from build123d import *

# Parameters (mm, degrees)
CUT_EXTRUDE1_DEPTH      = 16
CUT_EXTRUDE1_DEPTH_BACK = 16


with BuildPart() as part:
    # Sketch1 → Revolve1 (revolve)
    with BuildSketch(Plane.XY, mode=Mode.PRIVATE) as revolve1_sk:
        Polygon((7.91882362, 0), (6, 3.3235), (-6.3235, 3.3235), (-7, 4), (-7, 8), (30, 8), (30, 16), (35, 16), (35, 0), align=None)
    revolve(revolve1_sk.sketch.rotate(Axis((35, 0, 0), (-1, 0, 0)), 270), axis=Axis((35, 0, 0), (-1, 0, 0)))

    # Sketch2 → Cut-Extrude1 (cut, two sides: drawn at the far end of the back side and taken through both)
    with BuildSketch(Plane(origin=(0, 0, 0), x_dir=(1, 0, 0), z_dir=(0, 1, 0)).offset(-CUT_EXTRUDE1_DEPTH_BACK)):
        Polygon((-12, 12), (-12, -12), (4.5, -12), (-0.5, -7), (-7, -7), (-7, 7), (-0.5, 7), (4.5, 12), align=None)
    extrude(amount=CUT_EXTRUDE1_DEPTH + CUT_EXTRUDE1_DEPTH_BACK, mode=Mode.SUBTRACT)


solid = part.part
Could you check a few things on this model? Use its own coordinates, in mm. A direction names the side the tool comes from. Coordinates: 2 decimals unless noted, no trailing zeros. Write each loop counter-clockwise with the first axis right and the second up, starting at its lowest first coordinate (ties: lowest second). Pieces come first, ordered by that corner, then holes. Notation, with made-up numbers: (-9.5, 26.5) - (37.5, 26.5) arc R27 cw to (37.5, 49.5) - close; hole circle Ø6 at (60, -20). An arc over 180 degrees is marked (long way). Put each result on its own line as item: value. Start each with the question number.
Q1. I want a section at A-A on z = -5. Write out the boundary of the cut face in (x, y) (3 decimals).
Q2. Which directions (+Z, -Z, +X, -X, +Y, -Y) give clear straight access to the entire face, cutting with the end or side of a thin tool? Please do faces 1 (the flat face through (35, 0, 0)), 2 (the flat face through (-7, 4, 2)), 3 (the flat face through (-4, 0, 7)), 4 (the cylindrical face through (12, 0, -8)), 5 (the flat face through (-4, 0, -7)).
Q3. Thinking about a two-plate mould opening in Y: for faces 6 (the cylindrical face through (32.53, -15.62, -3.47)), 7 (the flat face through (30, 7.3, 3.8)), 8 (the cylindrical face through (-0.248, -3.244, -0.72)), which applies, pulls with the +Y half, pulls with the -Y half, needs draft (parallel to the pull), parting line crosses it, or undercut?
Q4. I want a section at D-D on y = -10.5. Write out the boundary of the cut face in (x, z), plus the area to 3 significant figures.
Q5. I want a section at C-C on x = 5.5. Write out the boundary of the cut face in (y, z).
Q6. I'm going to push flat-ended pins straight in: P1, Ø8, axis at x = 27, z = 10, coming from the -Y side; P2, Ø5, axis at x = -5.5, y = 0.5, coming from the +Z side; P3, Ø10, axis at x = 21.5, z = -3, coming from the -Y side; P4, Ø3, axis at y = 2, z = 2.5, coming from the -X side. Where does each tip first touch, or does it pass through?
Q7. I want a section at B-B on x = 31. Write out the boundary of the cut face in (y, z), plus the area to 3 significant figures.
Q8. Please list where these lines run through material, in increasing order: L1, parallel to Y at x = 0, z = 0; L2, parallel to X at y = 13.5, z = -2; L3, parallel to Z at x = -0.5, y = -7.
Checks:
1. outline: (-7, -6.245) - (30, -6.245) - (30, -15.199) - (35, -15.199) - (35, 15.199) - (30, 15.199) - (30, 6.245) - (-7, 6.245) - close
2. face 1: +Z, -Z, +X, +Y, -Y
2. face 2: +Z, -Z, -X, +Y, -Y
2. face 3: +Z, -X, +Y, -Y
2. face 4: -X
2. face 5: -Z, -X, +Y, -Y
3. face 6: parting line crosses it
3. face 7: needs draft
3. face 8: undercut
4. outline: (30, -12.07) - (35, -12.07) - (35, 12.07) - (30, 12.07) - close
4. area: 121 mm²
5. outline: circle Ø16 at (0, 0); hole circle Ø6.65 at (0, 0)
6. P1: y = -14.21
6. P2: z = 7
6. P3: y = -8
6. P4: x = -7
7. outline: circle Ø32 at (0, 0)
7. area: 804 mm²
8. L1: -8 to -3.32, 3.32 to 8
8. L2: 30 to 35
8. L3: -3.87 to 3.87
